Work out the finished part from the listing and answer in its coordinate system (mm). A direction names the side the tool comes from. Round coordinates to 2 decimals unless told otherwise and drop trailing zeros. Loops run counter-clockwise (first coordinate to the right, second up) from the corner with the lowest first, then second, coordinate; pieces in that order, holes last. Notation, with made-up numbers: (57.5, 3) -> (100.5, 3) arc R20 cw to (100.5, 9) -> close; hole circle Ø1 at (70, 29). An arc over 180 degrees is marked (long way). Write item = value, one per line. Start each with the question number.
```python
from build123d import *

# Parameters (mm, degrees)
BOSS_EXTRUDE1_DEPTH = 20


with BuildPart() as part:
    # Sketch1 → Boss-Extrude1 (new body)
    with BuildSketch(Plane.XY):
        with BuildLine():
            Line((0, 0), (605.341650479, 0))
            ThreePointArc((605.341650479, 0), (635.814099319, 6.980718334), (660.208845808, 26.53057538))
            Line((660.208845808, 26.53057538), (675, 45.2))
            Line((675, 45.2), (519.4, 170.9))
            Line((519.4, 170.9), (535.110173103, 190.347119609))
            Line((535.110173103, 190.347119609), (452.843320373, 255.524366816))
            ThreePointArc((452.843320373, 255.524366816), (312.777423466, 319.976650776), (158.75851208, 312.854339417))
            Line((158.75851208, 312.854339417), (139.1, 322.4))
            Line((139.1, 322.4), (-14.119827283, 6.856219748))
            Line((-14.119827283, 6.856219748), (0, 0))
        make_face()
    extrude(amount=BOSS_EXTRUDE1_DEPTH)


solid = part.part
```
Item 1: Section C-C (y = 229) is taken. Determine the outline of the cut face in (x, z).
Item 2: Flat-ended cylindrical pins translate along their axes: pin 1 (12 mm diameter, centred on x = 520.5, z = 7, fed in from +Y); pin 2 (8 mm diameter, centred on x = 102.5, z = 5, fed in from +Y); pin 3 (2 mm diameter, centred on x = 484, z = 10.5, fed in from +Y); pin 4 (10 mm diameter, centred on x = 89, y = 157, fed in from -Z). Find the tip coordinate at first contact, or state that the pin passes through.
Item 3: A tool of negligible diameter and unlimited length cuts with its end or side. For faces 1 (the flat face through (149.07, 317.56, 9.86)), 2 (the flat face through (63.563, 166.837, 9.86)), from which of +Z, -Z, +X, -X, +Y, -Y can it reach the whole face along a straight path? Write none if from no direction.
Item 4: The mould has two halves that part along Y. Classify faces 3 (the flat face through (527.145, 180.487, 9.86)), 4 (the flat face through (298, 0, 10)), 5 (the cylindrical face through (314.915, 319.553, 9.86)), 6 (the flat face through (326, 129, 20)): pulls with the +Y half, pulls with the -Y half, needs draft (parallel to the pull), parting line crosses it, or undercut.
Item 5: Section B-B (x = 51.5) is taken. Determine the outline of the cut face in (y, z).
Item 6: Section A-A (z = 11) is taken. Determine the outline of the cut face in (x, y), then the cut area to 3 significant figures.
Item 7: Find the intervals of material crossed by line 1 along Y through (x, z) = (582, 13.75); line 2 along X through (y, z) = (236, 1); line 3 along X through (y, z) = (212, 3), in increasing order. Write a range as [from, to].
Worked answers:
q1.outline = (93.75, 0) -> (486.32, 0) -> (486.32, 20) -> (93.75, 20) -> close
q2.pin_1 = 206.68
q2.pin_2 = 255.26
q2.pin_3 = 231.63
q2.pin_4 = 0
q3.face_1 = +Z, -Z, +Y
q3.face_2 = +Z, -Z, -X, +Y
q4.face_3 = undercut
q4.face_4 = pulls with the -Y half
q4.face_5 = pulls with the +Y half
q4.face_6 = needs draft
q5.outline = (0, 0) -> (141.99, 0) -> (141.99, 20) -> (0, 20) -> close
q6.outline = (-14.12, 6.86) -> (0, 0) -> (605.34, 0) arc R70 ccw to (660.21, 26.53) -> (675, 45.2) -> (519.4, 170.9) -> (535.11, 190.35) -> (452.84, 255.52) arc R326 ccw to (158.76, 312.85) -> (139.1, 322.4) -> close
q6.area = 154,000 mm2
q7.line_1 = [0, 120.33]
q7.line_2 = [97.15, 477.49]
q7.line_3 = [85.49, 507.78]
